Answer from the drawing. Dimensions are ordinates in mm from the lowest x, y and z of the part. Coordinates: 2 decimals unless noted, no trailing zeros. Loops run counter-clockwise (first coordinate to the right, second up) from the corner with the lowest first, then second, coordinate; pieces in that order, holes last.
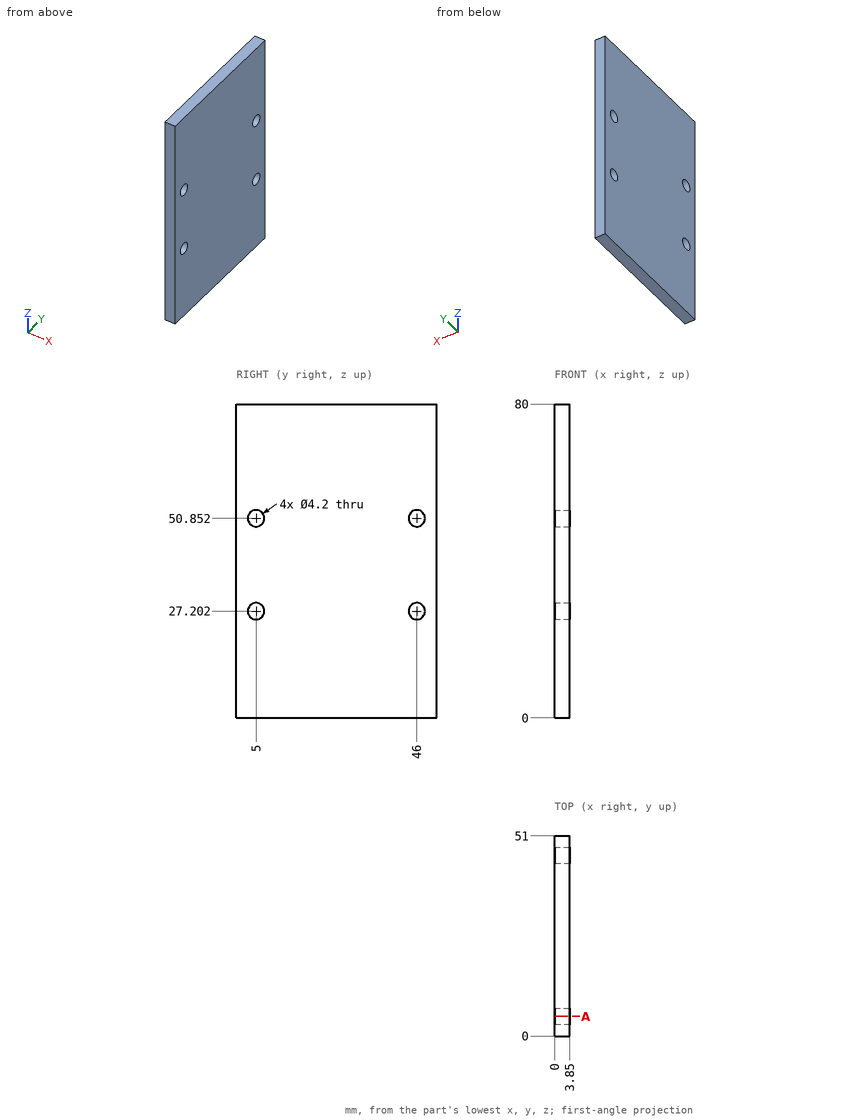
Item 1: Find the intervals of material crossed by line 1 along Z through (x, y) = (2.4, 46); line 2 along Y through (x, z) = (3.5, 51) (1 decimal); line 3 along Z through (x, y) = (2.6, 46.5), in increasing order.
Numbers:
line 1: z = 0 to 25.1, 29.3 to 48.75, 52.95 to 80
line 2: y = 0 to 2.9, 7.1 to 43.9, 48.1 to 51
line 3: z = 0 to 25.16, 29.24 to 48.81, 52.89 to 80
Item 2: Given pin 1 (1 mm diameter, centred on x = 2, y = 27, fed in from -Z); pin 2 (2.5 mm diameter, centred on y = 5, z = 27.2, fed in from -X), each flat-ended and moving along its own axis, determine where each tip first touches the part or whether it passes through.
Numbers:
pin 1: stops at z = 0
pin 2: passes through
Item 3: A cutting plane is placed at A-A on y = 5. Determine the outline of the cut face in (x, z).
Numbers:
outline: (0, 0) - (3.85, 0) - (3.85, 25.1) - (0, 25.1) - close; (0, 29.3) - (3.85, 29.3) - (3.85, 48.75) - (0, 48.75) - close; (0, 52.95) - (3.85, 52.95) - (3.85, 80) - (0, 80) - close
